Can you work these out from the drawing? Everything is in mm from the part's minimum corner. Round coordinates to 2 decimals unless told otherwise and drop trailing zeros. Loops run counter-clockwise (first coordinate to the right, second up) from the corner with the lowest first, then second, coordinate; pieces in that order, holes last. Notation, with made-up numbers: M 82,-26.75 L 127,-26.75 A23 cw 127,-10.75 Z; hole C 45,-36.5 d11. An arc over 180 degrees is marked long. Return JSON: item names as keys, results as strings. Group by question number.
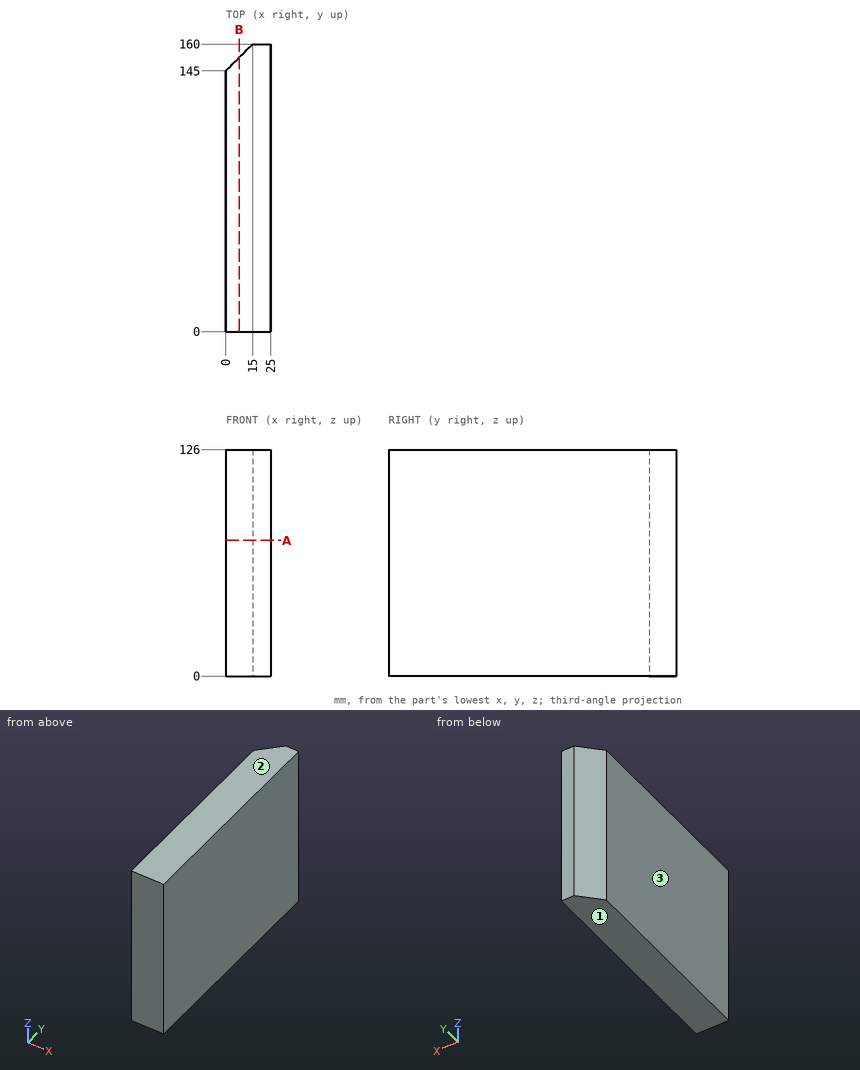
1. If we section it at B-B, the plane x = 7.5: Please give me the cut outline in (y, z).
2. I need wall thicknesses on probe 1 along Y at (x, z) = (1.5, 36); probe 2 along Y at (x, z) = (12.5, 32); probe 3 along X at (y, z) = (148, 79). Which ranges of each line are inside material? Lowest first, please.
3. We'd pull the mould along Z, two halves only. Please class the marked faces 1, 2 and 3: +Z half, -Z half, draft (parallel to the pull), parting line (faces both ways), or undercut.
4. If we section it at A-A, the plane z = 75.5: Please give me the cut outline in (x, y), then the cut area to 3 significant figures.
Geometry results:
{
 "1": {"outline": "M 0,0 L 152.5,0 L 152.5,126 L 0,126 Z"},
 "2": {"probe 1": "0 to 146.5", "probe 2": "0 to 157.5", "probe 3": "3 to 25"},
 "3": {"face 1": "-Z half", "face 2": "+Z half", "face 3": "draft"},
 "4": {"outline": "M 0,0 L 25,0 L 25,160 L 15,160 L 0,145 Z", "area": "3,890 mm^2"}
}
